The model under review builds one solid part; all positions refer to its coordinate system, in mm. A direction names the side the tool comes from. Give positions to 0.01 mm unless a question says otherwise; leave off trailing zeros. Order: outer loops, then holes, each group sorted by start corner. A loop starts at its lowest first (then second) coordinate and runs counter-clockwise, first axis right, second up. Notation, with made-up numbers: (35.5, 67) - (94.5, 67) arc R15 cw to (94.5, 80) - close; hole circle Ø4 at (78.25, 83.25). An arc over 180 degrees is marked (long way). Use CSV: the item, a comma, the result in double quotes. Start each with the question number.
1. For pin 1 (5 mm diameter, centred on x = 59, z = -4, fed in from +Y); pin 2 (3 mm diameter, centred on x = 26, y = 0, fed in from -Z); pin 3 (1 mm diameter, centred on x = 17.5, y = -3, fed in from -Z); pin 4 (3 mm diameter, centred on x = 5, y = 0, fed in from -Z), all flat-tipped, find the tip position at first contact; note any pin that passes through.
2. Take a section at C-C, the plane x = 46.5. State the section outline as (y, z) points, then the cut area to 3 significant figures.
3. Draft analysis for pull direction Y (two halves, no side actions). For faces 4 (the cylindrical face through (7.385, 0.751, -0.084)), 5 (the cylindrical face through (10.21, -0.59, -4.46)), 6 (the flat face through (11, 1.4, -4.5)), state which applies: released by +Y, released by -Y, zero draft, split by the parting line, or undercut.
4. Take a section at B-B, the plane z = 0. State the section outline as (x, y) points.
5. Machinability: for faces 1 (the flat face through (14, -1.42, 3.92)), 2 (the flat face through (9.4, -1.4, -4.5)), 3 (the flat face through (90, 0, 0)), which of the approach directions +Z, -Z, +X, -X, +Y, -Y give a long, thin tool a straight path to every point of the face, cutting with its end or side? Answer none if there is none.
6. Take a section at A-A, the plane y = 0. State the section outline as (x, z) points.
7. Take a section at D-D, the plane x = 5. State the section outline as (y, z) points.
8. To check wall thickness, follow line 1 (X direction, y = -5, z = -0.25); line 2 (X direction, y = 0, z = -0.5); line 3 (Y direction, x = 5, z = -3). State the ranges of each line that lie inside material, in increasing order. Write a range as [from, to].
```python
from build123d import *

# Parameters (mm, degrees)
CROSS_HOLE_DEPTH      = 91.39911504
CROSS_HOLE_DEPTH_BACK = 91.39911504
CROSS_HOLE_SKETCH_R   = 2.5


with BuildPart() as part:
    # Screw Profile Sketch → Screw Body Revolve (revolve)
    with BuildSketch(Plane.XY):
        Polygon((0, 0), (0, 6), (9.4, 6), (9.4, 4.5), (11, 4.5), (11, 6), (14, 6), (14, 4), (90, 4), (90, 0), align=None)
    revolve(axis=Axis((90, 0, 0), (-1, 0, 0)))

    # Cross Hole Sketch → Cross Hole (cut, two sides: drawn at the far end of the back side and taken through both)
    with BuildSketch(Plane.XY.offset(-CROSS_HOLE_DEPTH_BACK)):
        with Locations((5, 0)):
            Circle(CROSS_HOLE_SKETCH_R)
    extrude(amount=CROSS_HOLE_DEPTH + CROSS_HOLE_DEPTH_BACK, mode=Mode.SUBTRACT)


solid = part.part
```
Determined:
1,pin 1,"stops at y = 3.71"
1,pin 2,"stops at z = -4"
1,pin 3,"stops at z = -3.12"
1,pin 4,"passes through"
2,outline,"circle Ø8 at (0, 0)"
2,area,"50.3 mm²"
3,face 4,"undercut"
3,face 5,"split by the parting line"
3,face 6,"zero draft"
4,outline,"(0, -6) - (9.4, -6) - (9.4, -4.5) - (11, -4.5) - (11, -6) - (14, -6) - (14, -4) - (90, -4) - (90, 4) - (14, 4) - (14, 6) - (11, 6) - (11, 4.5) - (9.4, 4.5) - (9.4, 6) - (0, 6) - close; hole circle Ø5 at (5, 0)"
5,face 1,"+X"
5,face 2,"none"
5,face 3,"+Z, -Z, +X, +Y, -Y"
6,outline,"(0, -6) - (2.5, -6) - (2.5, 6) - (0, 6) - close; (7.5, -6) - (9.4, -6) - (9.4, -4.5) - (11, -4.5) - (11, -6) - (14, -6) - (14, -4) - (90, -4) - (90, 4) - (14, 4) - (14, 6) - (11, 6) - (11, 4.5) - (9.4, 4.5) - (9.4, 6) - (7.5, 6) - close"
7,outline,"(-2.5, -5.45) - (-2.5, 5.45) arc R6 ccw to start; (2.5, -5.45) arc R6 ccw to (2.5, 5.45) - close"
8,line 1,"x = [0, 9.4], [11, 14]"
8,line 2,"x = [0, 2.5], [7.5, 90]"
8,line 3,"y = [-5.2, -2.5], [2.5, 5.2]"
